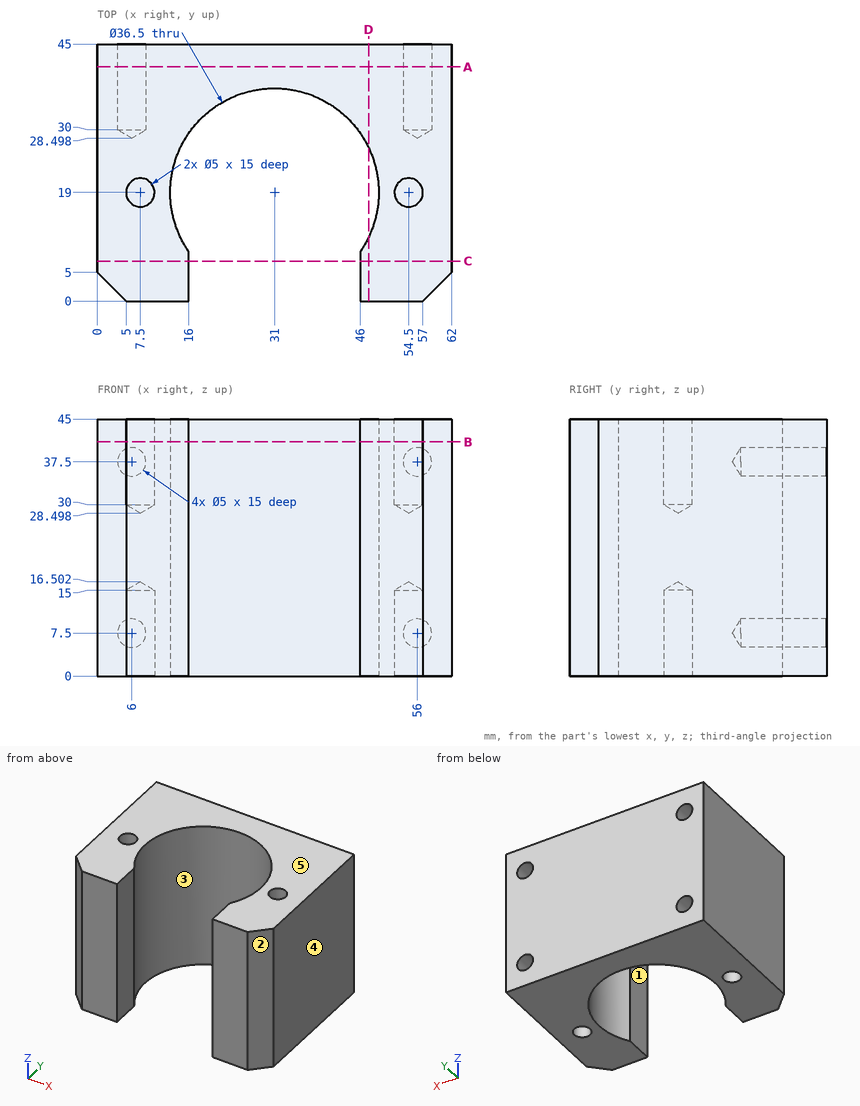
The drawing under review shows one solid part. Ordinate dimensions are in mm from its lowest x, y, z. A direction names the side the tool comes from. Give positions to 0.01 mm unless a question says otherwise; leave off trailing zeros. Write each loop counter-clockwise with the first axis right and the second up, starting at its lowest first coordinate (ties: lowest second). Pieces come first, ordered by that corner, then holes. Notation, with made-up numbers: (-4, 4) - (54, 4) arc R36 ccw to (54, 43) - close; hole circle Ø11 at (46, 59.25). An arc over 180 degrees is marked (long way). Answer in a Markdown table with one row per item. Add a question column.
1. Wall thickness on line 1 along X through (y, z) = (19, 5.5); line 2 along Z through (x, y) = (56, 41); line 3 along X through (y, z) = (42.25, 37.5): over which ranges is each line inside the solid? List them lowest first. Write a range as [from, to].
2. We need section A-A on y = 41. Write out the cut boundary in (x, z).
3. We need section B-B on z = 41. State how many separate pieces and enclosed holes the cut face has, then the cut area to 3 significant figures.
4. We need section C-C on y = 7. Write out the cut boundary in (x, z), then the cut area to 3 significant figures.
5. Draft analysis for pull direction X (two halves, no side actions). For the marked faces 3, 4 and 5, state which applies: +X half, -X half, draft (parallel to the pull), parting line (faces both ways), or undercut.
6. Tool access review of the marked faces 1 and 2: name each direction out of +Z, -Z, +X, -X, +Y, -Y from which nothing blocks a thin tool from reaching the whole face with its end or side.
7. We need section D-D on x = 47.5. Write out the cut boundary in (y, z).
8. Insertion check: P1, Ø4.5, axis at x = 56, z = 7.5, coming from the -Y side; P2, Ø4.5, axis at x = 54.5, y = 19, coming from the +Z side; P3, Ø4, axis at x = 56, z = 37.5, coming from the +Y side; P4, Ø4.5, axis at x = 7.5, y = 19, coming from the -Z side. Each pin has a flat end and moves straight along its axis. Give the tip position at first contact, or say it passes through.
Ans:
| question | item | result |
|---|---|---|
| 1 | line 1 | x = [0, 5], [10, 12.75], [49.25, 52], [57, 62] |
| 1 | line 2 | z = [0, 5], [10, 35], [40, 45] |
| 1 | line 3 | x = [0, 3.5], [8.5, 53.5], [58.5, 62] |
| 2 | outline | (0, 0) - (62, 0) - (62, 45) - (0, 45) - close; hole circle Ø5 at (6, 7.5); hole circle Ø5 at (6, 37.5); hole circle Ø5 at (56, 7.5); hole circle Ø5 at (56, 37.5) |
| 3 | separate pieces | 1 |
| 3 | enclosed holes | 2 |
| 3 | area | 1,590 mm^2 |
| 4 | outline | (0, 0) - (16, 0) - (16, 45) - (0, 45) - close; (46, 0) - (62, 0) - (62, 45) - (46, 45) - close |
| 4 | area | 1,440 mm^2 |
| 5 | face 3 | undercut |
| 5 | face 4 | +X half |
| 5 | face 5 | draft |
| 6 | face 1 | +Z, -Z, -Y |
| 6 | face 2 | +Z, -Z, +X, -Y |
| 7 | outline | (0, 0) - (11.2, 0) - (11.2, 45) - (0, 45) - close; (26.8, 0) - (45, 0) - (45, 45) - (26.8, 45) - close |
| 8 | P1 | stops at y = 0 |
| 8 | P2 | stops at z = 29.85 |
| 8 | P3 | stops at y = 29.7 |
| 8 | P4 | stops at z = 15.15 |
